Could you check a few things on this drawing? It's one solid part, dimensions in mm from its lowest x, y, z. A direction names the side the tool comes from. Coordinates: 2 decimals unless noted, no trailing zeros. Loops run counter-clockwise (first coordinate to the right, second up) from the corner with the lowest first, then second, coordinate; pieces in that order, holes last. Notation, with made-up numbers: (-1, -11.75) -> (56, -11.75) arc R9 cw to (56, -0.75) -> close; hole circle Ø9 at (12, 4.25). An arc over 180 degrees is marked (long way). One line per question, with ' | ' between items.
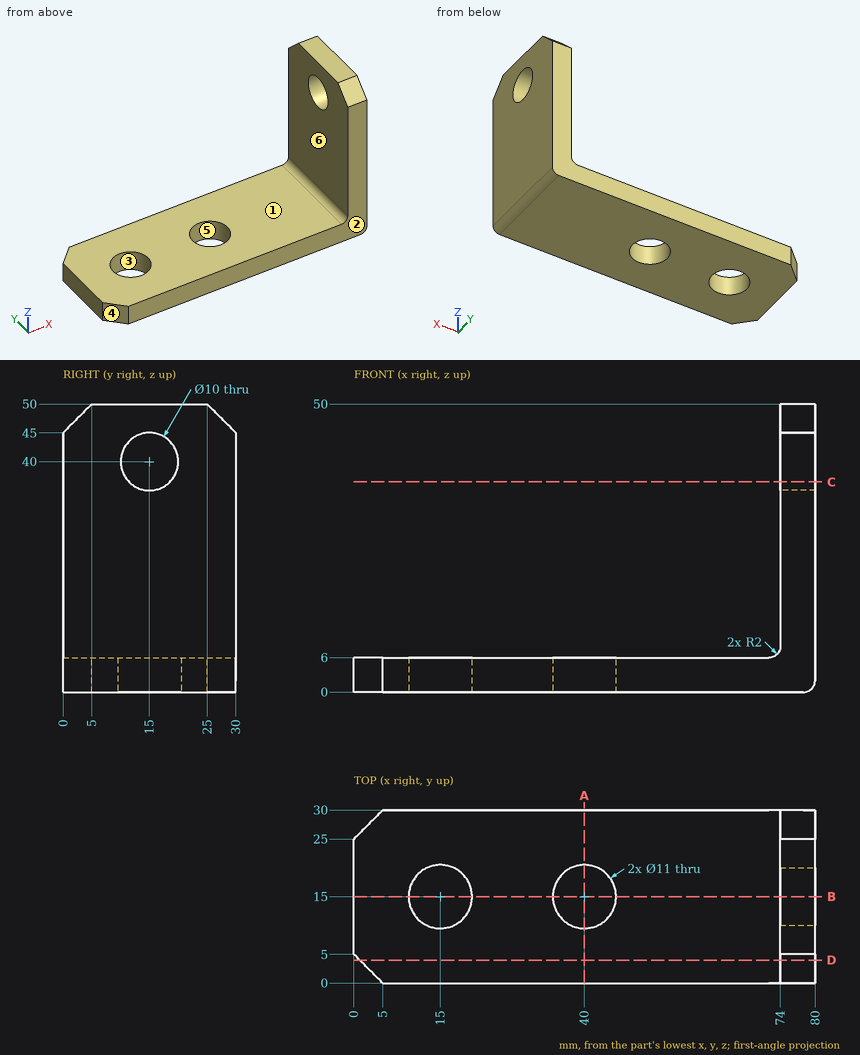
1) I need wall thicknesses on line 1 along Y through (x, z) = (15, 2.35); line 2 along Y through (x, z) = (77.4, 40); line 3 along X through (y, z) = (8, 20). Which ranges of each line are inside material? Lowest first, please. Write a range as from..to.
Data:
line 1: 0..9.5, 20.5..30 | line 2: 0..10, 20..30 | line 3: 74..80
2) We'd pull the mould along Y, two halves only. Please class the marked faces 3, 4, 5 and 6: pulls with the +Y half, pulls with the -Y half, needs draft (parallel to the pull), parting line crosses it, or undercut.
Data:
face 3: undercut | face 4: pulls with the -Y half | face 5: undercut | face 6: needs draft
3) If we section it at C-C on z = 36.5: Please give me the cut outline in (x, y).
Data:
outline: (74, 0) -> (80, 0) -> (80, 11.43) -> (74, 11.43) -> close; (74, 18.57) -> (80, 18.57) -> (80, 30) -> (74, 30) -> close
4) If we section it at A-A on x = 40: Please give me the cut outline in (y, z), and give its area (3 significant figures).
Data:
outline: (0, 0) -> (9.5, 0) -> (9.5, 6) -> (0, 6) -> close; (20.5, 0) -> (30, 0) -> (30, 6) -> (20.5, 6) -> close | area: 114 mm²
5) I'm going to push flat-ended pins straight in: pin 1 Ø15 at (x, y) = (44.5, 17.5) entering from +Z; pin 2 Ø10 at (x, y) = (15, 15) entering from -Z (3 decimals). Where does each tip first touch, or does it pass through?
Data:
pin 1: z = 6 | pin 2: through
6) If we section it at B-B on y = 15: Please give me the cut outline in (x, z).
Data:
outline: (0, 0) -> (9.5, 0) -> (9.5, 6) -> (0, 6) -> close; (20.5, 0) -> (34.5, 0) -> (34.5, 6) -> (20.5, 6) -> close; (45.5, 0) -> (78, 0) arc R2 ccw to (80, 2) -> (80, 35) -> (74, 35) -> (74, 8) arc R2 cw to (72, 6) -> (45.5, 6) -> close; (74, 45) -> (80, 45) -> (80, 50) -> (74, 50) -> close
7) If we section it at D-D on y = 4: Please give me the cut outline in (x, z), and give its area (3 significant figures).
Data:
outline: (1, 0) -> (78, 0) arc R2 ccw to (80, 2) -> (80, 49) -> (74, 49) -> (74, 8) arc R2 cw to (72, 6) -> (1, 6) -> close | area: 732 mm²
8) On a 3-axis mill with a long thin cutter (end or side, diameter ignored), from which of +Z, -Z, +X, -X, +Y, -Y can I reach the whole of each face in a straight line? I mean the marked faces 1 and 2. Say none if no direction works.
Data:
face 1: +Z, -X, +Y, -Y | face 2: +Z, -Z, +X, -X, -Y
